Part model, mm, in its own coordinate system. A direction names the side the tool comes from. Give positions to 0.01 mm unless a question says otherwise; leave off trailing zeros. Write each loop counter-clockwise with the first axis right and the second up, starting at its lowest first coordinate (ties: lowest second). Pieces come first, ordered by that corner, then holes.
```python
from build123d import *

# Parameters (mm, degrees)
SKETCH_2_R          = 2
CUT_EXTRUDE_1_DEPTH = 10


with BuildPart() as part:
    # 草图1 → 旋转1 (revolve)
    with BuildSketch(Plane.XY, mode=Mode.PRIVATE) as revolve_1_sk:
        Polygon((6, 3.693560261), (6, 0.693560261), (9, 0.693560261), (9, -7.306439739), (16, -7.306439739), (16, -13.306439739), (0, -13.306439739), (0, -9.306439739), (4, -9.306439739), (4, 3.693560261), align=None)
    revolve(revolve_1_sk.sketch.rotate(Axis((0, 0, 0), (0, 1, 0)), 90), axis=Axis((0, 0, 0), (0, 1, 0)))

    # 草图2 → 切除-拉伸1 (cut)
    with BuildSketch(Plane(origin=(0, 0, 0), x_dir=(0, 0, -1), z_dir=(1, 0, 0))):
        with Locations((0, -3.306439739)):
            Circle(SKETCH_2_R)
    extrude(amount=-CUT_EXTRUDE_1_DEPTH, mode=Mode.SUBTRACT)


solid = part.part
```
1) 3-axis set-ups, long thin cutter, end or side, ignore diameter. For faces 1 (the face through (-6.2, -3.22, 2)), 2 (the face through (7, -7.306, 7)), 3 (the face through (0, -13.306, 0)): which of +Z, -Z, +X, -X, +Y, -Y reach the whole face in a straight line?
Answers follow:
face 1: -X
face 2: +Y
face 3: +Z, -Z, +X, -X, -Y
2) Saw through at B-B, the plane x = 0. Write the cut outline in (y, z), then the cut area to 3 significant figures.
Answers follow:
outline: (-13.31, -16) - (-7.31, -16) - (-7.31, -9) - (0.69, -9) - (0.69, -6) - (3.69, -6) - (3.69, -4) - (-9.31, -4) - (-9.31, 4) - (3.69, 4) - (3.69, 6) - (0.69, 6) - (0.69, 9) - (-7.31, 9) - (-7.31, 16) - (-13.31, 16) - close
area: 268 mm2
3) Saw through at A-A, the plane z = 0. Write the cut outline in (x, y).
Answers follow:
outline: (-16, -13.31) - (16, -13.31) - (16, -7.31) - (9, -7.31) - (9, 0.69) - (6, 0.69) - (6, 3.69) - (4, 3.69) - (4, -9.31) - (-4, -9.31) - (-4, -5.31) - (-9, -5.31) - (-9, -7.31) - (-16, -7.31) - close; (-9, -1.31) - (-4, -1.31) - (-4, 3.69) - (-6, 3.69) - (-6, 0.69) - (-9, 0.69) - close
4) Saw through at C-C, the plane x = -6.5. Write the cut outline in (y, z).
Answers follow:
outline: (-13.31, -14.62) - (-7.31, -14.62) - (-7.31, -6.22) - (0.69, -6.22) - (0.69, 6.22) - (-7.31, 6.22) - (-7.31, 14.62) - (-13.31, 14.62) - close; hole circle Ø4 at (-3.31, 0)
5) Pin check, flat tips, straight feed: pin 1 Ø4 at (y, z) = (-3, 2.5) entering from -X; pin 2 Ø5 at (y, z) = (-3.31, 0) entering from +X; pin 3 Ø1.5 at (x, z) = (-2, -2) entering from +Y. Stop position of each tip, or through.
Answers follow:
pin 1: stops at x = -8.94
pin 2: stops at x = 9
pin 3: stops at y = -9.31
6) Wall check: L1, parallel to X at y = 0.75, z = 0; L2, parallel to X at y = 0, z = 0; L3, parallel to Y at x = -3, z = 0. Give the ranges that are in metal, low to high.
Answers follow:
L1: x = -6 to -4, 4 to 6
L2: x = -9 to -4, 4 to 9
L3: y = -13.31 to -9.31
7) Saw through at D-D, the plane y = -11.5. Write the cut outline in (x, z).
Answers follow:
outline: circle Ø32 at (0, 0)
8) Two-plate mould, pull along Z, no slides. Class faces 4 (the face through (0, -9.306, 0)), 5 (the face through (3.92, 3.694, -1.42)), 6 (the face through (15.62, -10.35, 3.47)): +Z half, -Z half, draft (parallel to the pull), parting line (faces both ways), or undercut.
Answers follow:
face 4: undercut
face 5: draft
face 6: parting line
